Here's how the part is built. I have some questions about the finished solid (model axes, mm). A direction names the side the tool comes from. Coordinates: 2 decimals unless noted, no trailing zeros. Write each loop counter-clockwise with the first axis right and the second up, starting at its lowest first coordinate (ties: lowest second). Pieces come first, ordered by that corner, then holes.
from build123d import *

# Parameters (mm, degrees)
BOSS_EXTRUDE1_DEPTH = 3
SKETCH2_R           = 5
CUT_EXTRUDE1_DEPTH  = 10
SKETCH4_W           = 3
SKETCH4_H           = 20
BOSS_EXTRUDE3_DEPTH = 3
SKETCH5_R           = 1
CUT_EXTRUDE2_DEPTH  = 10


with BuildPart() as part:
    # Sketch1 → Boss-Extrude1 (new body)
    with BuildSketch(Plane.XY):
        with BuildLine():
            Line((-16.33027103, 11.546525368), (25, 70))
            Line((25, 70), (25, 40))
            Line((25, 40), (19.854388756, -2.408992972))
            ThreePointArc((19.854388756, -2.408992972), (-7.196803073, -18.660279353), (-16.33027103, 11.546525368))
        make_face()
    extrude(amount=-BOSS_EXTRUDE1_DEPTH)

    # Sketch2 → Cut-Extrude1 (cut)
    with BuildSketch(Plane.XY):
        Circle(SKETCH2_R)
    extrude(amount=-CUT_EXTRUDE1_DEPTH, mode=Mode.SUBTRACT)

    # Sketch4 → Boss-Extrude3 (add)
    with BuildSketch(Plane(origin=(25, 0, 0), x_dir=(0, 0, -1), z_dir=(1, 0, 0))):
        with Locations((1.5, 55)):
            Rectangle(SKETCH4_W, SKETCH4_H)
    extrude(amount=BOSS_EXTRUDE3_DEPTH)

    # Sketch5 → Cut-Extrude2 (cut)
    with BuildSketch(Plane.XY):
        with Locations((0, 16.5)):
            Circle(SKETCH5_R)
        with Locations((0, -16.5)):
            Circle(SKETCH5_R)
        with Locations((16.5, 0)):
            Circle(SKETCH5_R)
        with Locations((-16.5, 0)):
            Circle(SKETCH5_R)
    extrude(amount=-CUT_EXTRUDE2_DEPTH, mode=Mode.SUBTRACT)


solid = part.part
1. I want a section at A-A (z = -0.7). List the corners of the cut face in (x, y) for me.
2. If I drill on line 1 (Y direction, x = -0.5, z = -0.6); line 2 (Y direction, x = 0, z = -1.8); line 3 (Y direction, x = -3.5, z = -1.1), over which ranges is the centre line in solid material (lowest first)?
3. For pin 1 Ø2.5 at (x, y) = (16.5, 0) entering from -Z; pin 2 Ø1 at (y, z) = (34, -1) entering from +X; pin 3 Ø5 at (x, y) = (4.5, 48) entering from +Z; pin 4 Ø1.5 at (y, z) = (43.5, -2) entering from +X, each with a flat end and sliding along its axis, tell me the tip position at first contact or that it passes through.
4. I want a section at B-B (y = -16.5). List the corners of the cut face in (x, z) for me, then the cut area to 3 significant figures.
5. Thinking about a two-plate mould opening in Y: for faces 4 (the face through (-0.217, 15.524, -1.479)), 5 (the face through (-6.72, -18.837, -1.479)), 6 (the face through (17.424, -0.383, -1.479)), 7 (the face through (4, 16, -3)), which applies, pulls with the +Y half, pulls with the -Y half, needs draft (parallel to the pull), parting line crosses it, or undercut?
6. On a 3-axis mill with a long thin cutter (end or side, diameter ignored), from which of +Z, -Z, +X, -X, +Y, -Y can I reach the whole of each face in a straight line? I mean faces 1 (the face through (26, 45, -1)), 2 (the face through (4, 16, 0)), 3 (the face through (26, 65, -1)). Say none if no direction works.
7. I want a section at C-C (x = 0). List the corners of the cut face in (y, z) for me.
8. I want a section at D-D (x = 16.5). List the corners of the cut face in (y, z) for me.
Response values:
1. outline: (-16.33, 11.55) arc R20 ccw (long way) to (19.85, -2.41) - (25, 40) - (25, 45) - (28, 45) - (28, 65) - (25, 65) - (25, 70) - close; hole circle Ø2 at (-16.5, 0); hole circle Ø10 at (0, 0); hole circle Ø2 at (0, -16.5); hole circle Ø2 at (0, 16.5); hole circle Ø2 at (16.5, 0)
2. line 1: y = -19.99 to -17.37, -15.63 to -4.97, 4.97 to 15.63, 17.37 to 33.94
2. line 2: y = -20 to -17.5, -15.5 to -5, 5 to 15.5, 17.5 to 34.64
2. line 3: y = -19.69 to -3.57, 3.57 to 29.69
3. pin 1: stops at z = -3
3. pin 2: stops at x = 24.33
3. pin 3: passes through
3. pin 4: stops at x = 25
4. outline: (-11.3, -3) - (-1, -3) - (-1, 0) - (-11.3, 0) - close; (1, -3) - (11.3, -3) - (11.3, 0) - (1, 0) - close
4. area: 61.8 mm2
5. face 4: undercut
5. face 5: parting line crosses it
5. face 6: undercut
5. face 7: needs draft
6. face 1: +Z, -Z, +X, -Y
6. face 2: +Z, +X, -X, +Y, -Y
6. face 3: +Z, -Z, +X, +Y
7. outline: (-20, -3) - (-17.5, -3) - (-17.5, 0) - (-20, 0) - close; (-15.5, -3) - (-5, -3) - (-5, 0) - (-15.5, 0) - close; (5, -3) - (15.5, -3) - (15.5, 0) - (5, 0) - close; (17.5, -3) - (34.64, -3) - (34.64, 0) - (17.5, 0) - close
8. outline: (-11.3, -3) - (-1, -3) - (-1, 0) - (-11.3, 0) - close; (1, -3) - (57.98, -3) - (57.98, 0) - (1, 0) - close
